from build123d import *

# Parameters (mm, degrees)
SKETCH1_W           = 50
SKETCH1_H           = 50
SKETCH1_W_2         = 46
SKETCH1_H_2         = 46
BOSS_EXTRUDE1_DEPTH = 194.4


with BuildPart() as part:
    # Sketch1 → Boss-Extrude1 (new body)
    with BuildSketch(Plane.XY):
        Rectangle(SKETCH1_W, SKETCH1_H)
        Rectangle(SKETCH1_W_2, SKETCH1_H_2, mode=Mode.SUBTRACT)
    extrude(amount=BOSS_EXTRUDE1_DEPTH)


solid = part.part
CAD build for the part. Positions are in the model's coordinates, mm. A direction names the side the tool comes from. Round coordinates to 2 decimals unless told otherwise and drop trailing zeros. Write each loop counter-clockwise with the first axis right and the second up, starting at its lowest first coordinate (ties: lowest second). Pieces come first, ordered by that corner, then holes. Notation, with made-up numbers: (12.25, 53) -> (23.25, 53) arc R20 cw to (23.25, 91) -> close; hole circle Ø6 at (33.25, 33). An arc over 180 degrees is marked (long way). Answer as a JSON object with one key per item and string values.
(1) Band-saw the part on A-A, the plane x = 1. List the corners of the cut face in (y, z).
Reported:
{"outline": "(-25, 0) -> (-23, 0) -> (-23, 194.4) -> (-25, 194.4) -> close; (23, 0) -> (25, 0) -> (25, 194.4) -> (23, 194.4) -> close"}
(2) Probe probe 1 along Y at (x, z) = (2.5, 155.5). List the from-to ranges inside material, lowest first. Write a range as [from, to].
Reported:
{"probe 1": "y = [-25, -23], [23, 25]"}
(3) Two-plate mould, pull along X, no slides. Class faces 1 (the face through (-2, -24, 194.4)), 2 (the face through (-25, 0, 96)), 3 (the face through (-23, 0, 96)): +X half, -X half, draft (parallel to the pull), parting line (faces both ways), or undercut.
Reported:
{"face 1": "draft", "face 2": "-X half", "face 3": "undercut"}
(4) Which spindle directions (+Z, -Z, +X, -X, +Y, -Y) get a long thin tool onto all of the face, cutting with end or side? Do faces 4 (the face through (-2, -24, 0)), 5 (the face through (23, 0, 96)). Say none if no direction does.
Reported:
{"face 4": "-Z, +X, -X, +Y, -Y", "face 5": "+Z, -Z"}
(5) Band-saw the part on B-B, the plane z = 107. List the corners of the cut face in (x, y), then the cut area to 3 significant figures.
Reported:
{"outline": "(-25, -25) -> (25, -25) -> (25, 25) -> (-25, 25) -> close; hole (-23, -23) -> (23, -23) -> (23, 23) -> (-23, 23) -> close", "area": "384 mm^2"}
